Here's how the part is built. I have some questions about the finished solid (model axes, mm). Give positions to 0.01 mm unless a question says otherwise; leave off trailing zeros. Write each loop counter-clockwise with the first axis right and the second up, starting at its lowest first coordinate (ties: lowest second). Pieces come first, ordered by that corner, then holes. Notation, with made-up numbers: (78, -8) - (83, -8) arc R8 ccw to (83, -1) - close; hole circle Ø6 at (25, 79). An arc over 180 degrees is marked (long way). One line per item, written item: value. Start each with the question number.
1) Imagine slicing it at A-A on x = 0. Write out the boundary of the cut face in (y, z).
2) Imagine slicing it at C-C on y = 26.5. Write out the boundary of the cut face in (x, z).
3) Imagine slicing it at B-B on z = 13.5. Write out the boundary of the cut face in (x, y), plus the area to 3 significant figures.
4) I'm going to push flat-ended pins straight in: P1, Ø6, axis at x = 35, z = 7.5, coming from the +Y side; P2, Ø4, axis at x = 35, z = 7.5, coming from the +Y side. Where does each tip first touch, or does it pass through?
5) Please list where these lines run through material, in increasing order: L1, parallel to X at y = 0, z = 9; L2, parallel to Z at x = 35, y = 18; L3, parallel to X at y = 8, z = 11.5. Write a range as [from, to].
6) Imagine slicing it at D-D on y = -24.5. Write out the boundary of the cut face in (x, z).
from build123d import *

# Parameters (mm, degrees)
SKETCH_1_W                   = 90
SKETCH_1_H                   = 60
EXTRUDE_1_DEPTH              = 15
SKETCH_3_R                   = 8
CUT_EXTRUDE_1_DEPTH          = 57.124860802
SKETCH_4_W                   = 5
SKETCH_4_H                   = 5.148629024
CUT_EXTRUDE_2_DEPTH          = 20
HOLE_WIZARD_M5_1_D           = 4.2
HOLE_WIZARD_M5_1_DEPTH       = 12.4
HOLE_WIZARD_M5_1_CSINK_D     = 5.05
HOLE_WIZARD_M5_1_CSINK_ANGLE = 92
HOLE_WIZARD_M5_1_TIP         = 1.2618073
SKETCH_8_R                   = 2
CUT_EXTRUDE_4_DEPTH          = 10
HOLE_WIZARD_M6_1_D           = 5
HOLE_WIZARD_M6_1_DEPTH       = 15
HOLE_WIZARD_M6_1_CSINK_D     = 6.05
HOLE_WIZARD_M6_1_CSINK_ANGLE = 92
HOLE_WIZARD_M6_1_TIP         = 1.502151548
HOLE_WIZARD_M6_2_D           = 5
HOLE_WIZARD_M6_2_DEPTH       = 15
HOLE_WIZARD_M6_2_CSINK_D     = 6.05
HOLE_WIZARD_M6_2_CSINK_ANGLE = 92
HOLE_WIZARD_M6_2_TIP         = 1.502151548
CHAMFER_2_SIZE               = 0.5
CHAMFER_3_SIZE               = 0.5


with BuildPart() as part:
    # 草图1 → 凸台-拉伸1 (new body)
    with BuildSketch(Plane.XY):
        Rectangle(SKETCH_1_W, SKETCH_1_H)
    extrude(amount=EXTRUDE_1_DEPTH)

    # 草图3 → 切除-拉伸1 (cut, through all)
    with BuildSketch(Plane.XY.offset(15)):
        Circle(SKETCH_3_R)
    extrude(amount=-CUT_EXTRUDE_1_DEPTH, mode=Mode.SUBTRACT)

    # 草图4 → 切除-拉伸2 (cut)
    with BuildSketch(Plane.XY.offset(15)):
        with Locations((0, 7.574314512)):
            Rectangle(SKETCH_4_W, SKETCH_4_H)
    extrude(amount=-CUT_EXTRUDE_2_DEPTH, mode=Mode.SUBTRACT)

    # M5 螺纹孔1
    with Locations(Plane.XY.offset(15)):
        with Locations((15, 0), (-15, 0)):
            CounterSinkHole(HOLE_WIZARD_M5_1_D / 2, HOLE_WIZARD_M5_1_CSINK_D / 2, depth=HOLE_WIZARD_M5_1_DEPTH, counter_sink_angle=HOLE_WIZARD_M5_1_CSINK_ANGLE)
            with Locations((0, 0, -(HOLE_WIZARD_M5_1_DEPTH + HOLE_WIZARD_M5_1_TIP / 2))):  # 118° drill point
                Cone(0, HOLE_WIZARD_M5_1_D / 2, HOLE_WIZARD_M5_1_TIP, mode=Mode.SUBTRACT)

    # 草图8 → 切除-拉伸4 (cut)
    with BuildSketch(Plane.XZ.offset(30)):
        with Locations(Location((-23, 7.5, 0), (0, 0, 270))):
            Circle(SKETCH_8_R)
        with Locations(Location((23, 7.5, 0), (0, 0, 270))):
            Circle(SKETCH_8_R)
    extrude(amount=-CUT_EXTRUDE_4_DEPTH, mode=Mode.SUBTRACT)

    # M6 螺纹孔1
    with Locations(Plane(origin=(0, 30, 0), x_dir=(1, 0, 0), z_dir=(0, 1, 0))):
        with Locations((-35, -7.5), (35, -7.5)):
            CounterSinkHole(HOLE_WIZARD_M6_1_D / 2, HOLE_WIZARD_M6_1_CSINK_D / 2, depth=HOLE_WIZARD_M6_1_DEPTH, counter_sink_angle=HOLE_WIZARD_M6_1_CSINK_ANGLE)
            with Locations((0, 0, -(HOLE_WIZARD_M6_1_DEPTH + HOLE_WIZARD_M6_1_TIP / 2))):  # 118° drill point
                Cone(0, HOLE_WIZARD_M6_1_D / 2, HOLE_WIZARD_M6_1_TIP, mode=Mode.SUBTRACT)

    # M6 螺纹孔2
    with Locations(Plane(origin=(0, -30, 0), x_dir=(-1, 0, 0), z_dir=(0, -1, 0))):
        with Locations((35, -7.5), (-35, -7.5)):
            CounterSinkHole(HOLE_WIZARD_M6_2_D / 2, HOLE_WIZARD_M6_2_CSINK_D / 2, depth=HOLE_WIZARD_M6_2_DEPTH, counter_sink_angle=HOLE_WIZARD_M6_2_CSINK_ANGLE)
            with Locations((0, 0, -(HOLE_WIZARD_M6_2_DEPTH + HOLE_WIZARD_M6_2_TIP / 2))):  # 118° drill point
                Cone(0, HOLE_WIZARD_M6_2_D / 2, HOLE_WIZARD_M6_2_TIP, mode=Mode.SUBTRACT)

    # 倒角2
    chamfer_2_edges = [part.edges().sort_by_distance(p)[0] for p in [
        (-45, 0, 15),
        (0, -30, 15),
        (45, 0, 15),
        (0, -30, 0),
        (-45, 0, 0),
        (0, 30, 0),
        (45, 0, 0),
        (0, 30, 15),
        (45, -30, 7.5),
        (-45, -30, 7.5),
        (-45, 30, 7.5),
        (45, 30, 7.5),
    ]]
    chamfer(chamfer_2_edges, length=CHAMFER_2_SIZE)

    # 倒角3
    chamfer_3_edges = [part.edges().sort_by_distance(p)[0] for p in [
        (0, -8, 0),
        (0, -8, 15),
        (0, 10.148629024, 0),
        (-2.5, 8.87398555, 0),
        (2.5, 8.87398555, 0),
        (-2.5, 8.87398555, 15),
        (2.5, 8.87398555, 15),
        (0, 10.148629024, 15),
    ]]
    chamfer(chamfer_3_edges, length=CHAMFER_3_SIZE)


solid = part.part
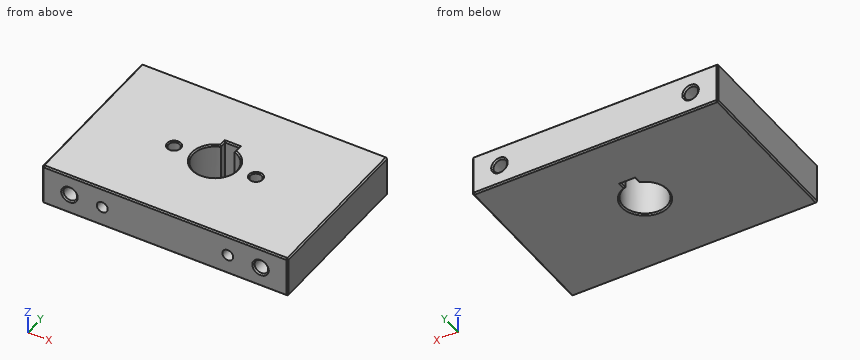
Numbers:
1. outline: (-30, 0.5) - (-29.5, 0) - (-8.5, 0) - (-8, 0.5) - (-8, 14.5) - (-8.5, 15) - (-29.5, 15) - (-30, 14.5) - close; (10.15, 0.5) - (10.65, 0) - (29.5, 0) - (30, 0.5) - (30, 14.5) - (29.5, 15) - (10.65, 15) - (10.15, 14.5) - close
2. outline: (-45, 0.5) - (-44.5, 0) - (44.5, 0) - (45, 0.5) - (45, 14.5) - (44.5, 15) - (-44.5, 15) - (-45, 14.5) - close; hole circle Ø5 at (-35, 7.5); hole circle Ø5 at (35, 7.5)
3. outline: (-45, -29.5) - (-44.5, -30) - (44.5, -30) - (45, -29.5) - (45, 29.5) - (44.5, 30) - (-44.5, 30) - (-45, 29.5) - close; hole circle Ø4.2 at (-15, 0); hole (-2.5, 7.6) arc R8 ccw (long way) to (2.5, 7.6) - (2.5, 10.15) - (-2.5, 10.15) - close; hole circle Ø4.2 at (15, 0)
3. area: 5,160 mm^2
4. P1: y = 29.98
4. P2: y = 14.7
5. L1: [-45, -17.1], [-12.9, -8], [8, 12.9], [17.1, 45]
5. L2: [0, 5], [10, 15]
5. L3: [-45, -2.5], [2.5, 45]
6. outline: (-45, 0.5) - (-44.5, 0) - (44.5, 0) - (45, 0.5) - (45, 14.5) - (44.5, 15) - (-44.5, 15) - (-45, 14.5) - close; hole circle Ø5 at (-35, 7.5); hole circle Ø4 at (-23, 7.5); hole circle Ø4 at (23, 7.5); hole circle Ø5 at (35, 7.5)
